Study the drawing (mm; zero at the part's minimum x, y, z) and answer. A direction names the side the tool comes from. Coordinates: 2 decimals unless noted, no trailing zeros. Order: outer loops, then holes, each group sorted by start corner. A loop starts at its lowest first (then second) coordinate and runs counter-clockwise, first axis right, second up. Notation, with made-up numbers: M 14.5,-39.75 L 72.5,-39.75 A27 ccw 72.5,-6.75 Z; hole C -28,11 d4. An arc over 180 degrees is marked long. Put each result on its own line as item: value.
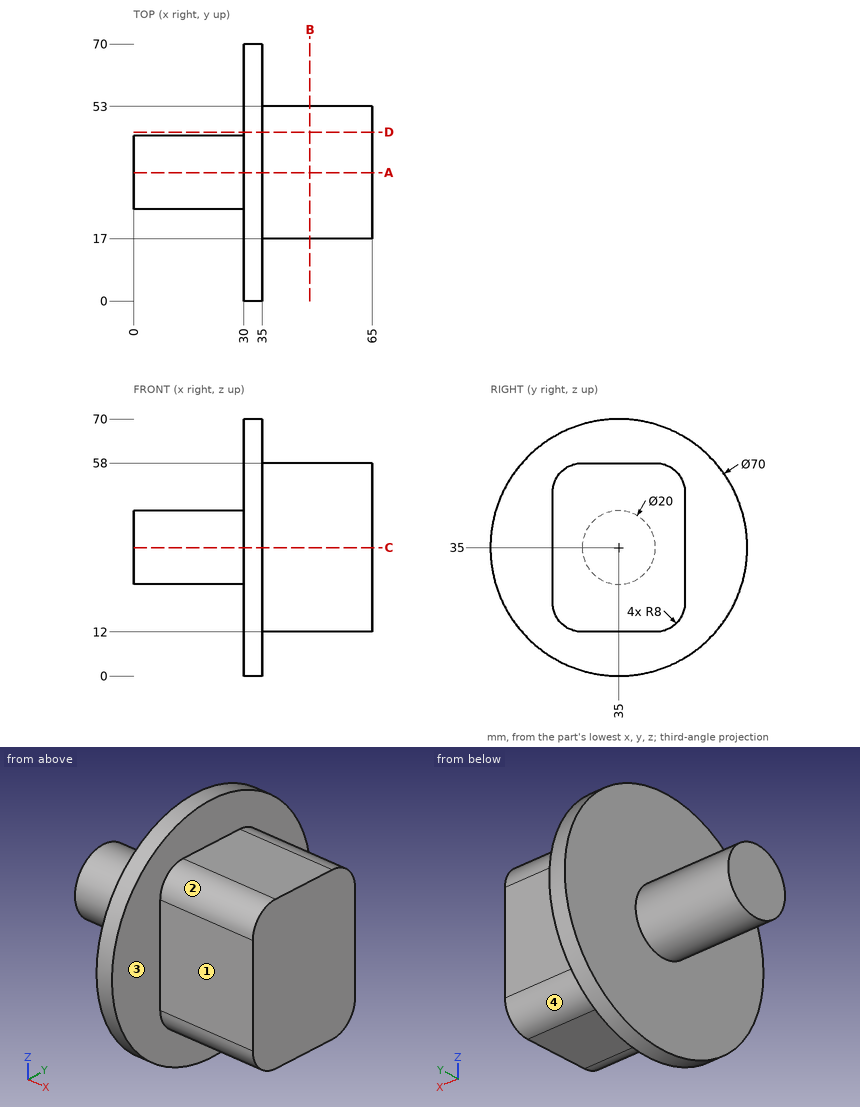
Q1. Consider line 1 along Y through (x, z) = (37, 27.5); line 2 along X through (y, z) = (25, 64.5); line 3 along Z through (x, y) = (45, 40). Determine where each line is inside the solid, lowest interval first.
Answers below:
line 1: y = 17 to 53
line 2: x = 30 to 35
line 3: z = 12 to 58
Q2. Given pin 1 (6 mm diameter, centred on x = 53.5, y = 37.5, fed in from +Z); pin 2 (5 mm diameter, centred on y = 51.5, z = 39.5, fed in from -X); pin 3 (24 mm diameter, centred on x = 51.5, z = 42, fed in from +Y); pin 4 (1.5 mm diameter, centred on x = 36, z = 61, fed in from -Y), each flat-ended and moving along its own axis, determine where each tip first touches the part or whether it passes through.
Answers below:
pin 1: stops at z = 58
pin 2: stops at x = 30
pin 3: stops at y = 53
pin 4: passes through
Q3. Find section C-C on z = 35. Write down the section's boundary in (x, y).
Answers below:
outline: M 0,25 L 30,25 L 30,0 L 35,0 L 35,17 L 65,17 L 65,53 L 35,53 L 35,70 L 30,70 L 30,45 L 0,45 Z
Q4. Find section A-A on y = 35. Write down the section's boundary in (x, z).
Answers below:
outline: M 0,25 L 30,25 L 30,0 L 35,0 L 35,12 L 65,12 L 65,58 L 35,58 L 35,70 L 30,70 L 30,45 L 0,45 Z
Q5. A tool of negligible diameter and unlimited length cuts with its end or side. For the marked faces 1, 2, 3 and 4, from which of +Z, -Z, +X, -X, +Y, -Y can it reach the whole face along a straight path? Write none if from no direction.
Answers below:
face 1: +Z, -Z, +X, -Y
face 2: +Z, +X, -Y
face 3: +X
face 4: -Z, +X, +Y
Q6. Find section D-D on y = 46. Write down the section's boundary in (x, z), plus the area to 3 significant figures.
Answers below:
outline: M 30,1.77 L 35,1.77 L 35,12.06 L 65,12.06 L 65,57.94 L 35,57.94 L 35,68.23 L 30,68.23 Z
area: 1,710 mm^2
Q7. Find section B-B on x = 48. Write down the section's boundary in (y, z), plus the area to 3 significant figures.
Answers below:
outline: M 17,20 A8 ccw 25,12 L 45,12 A8 ccw 53,20 L 53,50 A8 ccw 45,58 L 25,58 A8 ccw 17,50 Z
area: 1,600 mm^2
